Geometry check sheet. Reference: drawing and pictorial views, mm from the part's lowest x, y, z. A direction names the side the tool comes from. Round coordinates to 2 decimals unless told otherwise and drop trailing zeros. Write each loop counter-clockwise with the first axis right and the second up, starting at its lowest first coordinate (ties: lowest second). Pieces come first, ordered by that corner, then holes. Notation, with made-up numbers: (52.25, 83.5) -> (65.25, 83.5) arc R28 cw to (65.25, 108.5) -> close; hole circle Ø8 at (89.25, 88). An arc over 180 degrees is marked (long way). Answer as a JSON object with one key per item and string values. Group by question number.
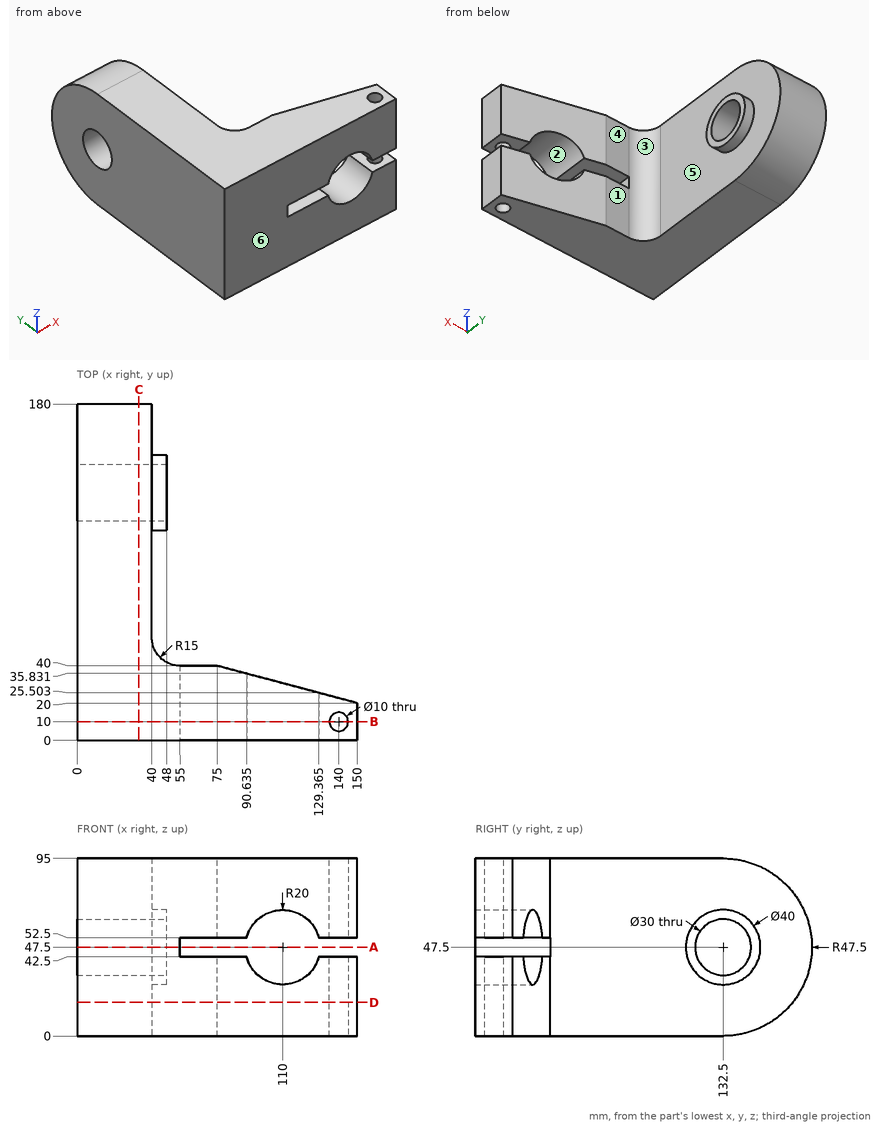
(1) Access from +Z, -Z, +X, -X, +Y, -Y to the whole of each face (thin tool, end or side, straight path). Record for the marked faces 1, 2 and 3.
(2) Go/stop test with flat-tipped pins: pin 1 Ø3 at (x, z) = (98, 18) entering from +Y; pin 2 Ø6 at (x, z) = (70, 25.5) entering from +Y; pin 3 Ø2 at (x, z) = (123.5, 80.5) entering from +Y. Record where each tip stops, or that it passes through.
(3) Scan lines: line 1 along X through (y, z) = (87, 14); line 2 along Z through (x, y) = (31, 132.5). Record each from-to range of solid material in increasing order.
(4) Release check for a two-part mould opening along Y. For the marked faces 4, 5 and 6 record: pulls with the +Y half, pulls with the -Y half, needs draft (parallel to the pull), parting line crosses it, or undercut.
(5) Section check B-B on y = 10. Record the cut outline in (x, z) (1 decimal).
(6) Section check D-D on z = 18. Record the cut outline in (x, y), then the cut area to 3 significant figures.
(7) Section check C-C on x = 33. Record the cut outline in (y, z).
(8) Section check A-A on z = 47.5. Record the cut outline in (x, y), then the cut area to 3 significant figures.
Data:
{
 "1": {"face 1": "+Z, -Z, +X, +Y", "face 2": "+Y, -Y", "face 3": "+Z, -Z, +X"},
 "2": {"pin 1": "stops at y = 34.27", "pin 2": "stops at y = 40", "pin 3": "stops at y = 27.33"},
 "3": {"line 1": "x = 0 to 40", "line 2": "z = 0 to 32.5, 62.5 to 95"},
 "4": {"face 4": "pulls with the +Y half", "face 5": "undercut", "face 6": "pulls with the -Y half"},
 "5": {"outline": "(0, 0) -> (135, 0) -> (135, 42.5) -> (129.4, 42.5) arc R20 cw to (90.6, 42.5) -> (55, 42.5) -> (55, 52.5) -> (90.6, 52.5) arc R20 cw to (129.4, 52.5) -> (135, 52.5) -> (135, 95) -> (0, 95) -> close; (145, 0) -> (150, 0) -> (150, 42.5) -> (145, 42.5) -> close; (145, 52.5) -> (150, 52.5) -> (150, 95) -> (145, 95) -> close"},
 "6": {"outline": "(0, 0) -> (150, 0) -> (150, 20) -> (75, 40) -> (55, 40) arc R15 cw to (40, 55) -> (40, 169.73) -> (0, 169.73) -> close; hole circle Ø10 at (140, 10)", "area": "10,400 mm²"},
 "7": {"outline": "(0, 0) -> (132.5, 0) arc R47.5 ccw to (132.5, 95) -> (0, 95) -> close; hole circle Ø30 at (132.5, 47.5)"},
 "8": {"outline": "(0, 0) -> (55, 0) -> (55, 40) arc R15 cw to (40, 55) -> (40, 112.5) -> (48, 112.5) -> (48, 117.5) -> (0, 117.5) -> close; (0, 147.5) -> (48, 147.5) -> (48, 152.5) -> (40, 152.5) -> (40, 180) -> (0, 180) -> close", "area": "6,730 mm²"}
}
